from build123d import *

# Parameters (mm, degrees)
SKETCH_1_W             = 90
SKETCH_1_H             = 75
SKETCH_1_R             = 26
EXTRUDE_1_DEPTH        = 30
HOLE_WIZARD_M8_1_D     = 6.8
HOLE_WIZARD_M8_1_DEPTH = 19.75
HOLE_WIZARD_M8_1_TIP   = 2.042926105
CHAMFER_1_SIZE         = 15
HOLE_WIZARD_M8_2_D     = 6.8
HOLE_WIZARD_M8_2_DEPTH = 19.75
HOLE_WIZARD_M8_2_TIP   = 2.042926105


with BuildPart() as part:
    # 草图1 → 凸台-拉伸1 (new, symmetric)
    with BuildSketch(Plane.XY):
        with Locations((0, 5)):
            Rectangle(SKETCH_1_W, SKETCH_1_H)
        Circle(SKETCH_1_R, mode=Mode.SUBTRACT)
    extrude(amount=EXTRUDE_1_DEPTH, both=True)

    # M8 螺纹孔1
    with Locations(Plane(origin=(-32.5, 0, 30), x_dir=(1, 0, 0), z_dir=(0, 0, 1))):
        with Locations((0, 0), (9.519029611, 22.980970389), (9.519029611, -22.980970389), (55.480970389, -22.980970389), (65, 0), (55.480970389, 22.980970389)):
            Hole(HOLE_WIZARD_M8_1_D / 2, depth=HOLE_WIZARD_M8_1_DEPTH)
            with Locations((0, 0, -(HOLE_WIZARD_M8_1_DEPTH + HOLE_WIZARD_M8_1_TIP / 2))):  # 118° drill point
                Cone(0, HOLE_WIZARD_M8_1_D / 2, HOLE_WIZARD_M8_1_TIP, mode=Mode.SUBTRACT)

    # 倒角1
    chamfer_1_edges = [part.edges().sort_by_distance(p)[0] for p in [
        (45, -32.5, 0),
        (-45, -32.5, 0),
    ]]
    chamfer(chamfer_1_edges, length=CHAMFER_1_SIZE)

    # M8 螺纹孔2
    with Locations(Plane(origin=(32.5, 42.5, -20), x_dir=(1, 0, 0), z_dir=(0, 1, 0))):
        with Locations((0, 0), (0, -40), (-65, -40), (-65, 0)):
            Hole(HOLE_WIZARD_M8_2_D / 2, depth=HOLE_WIZARD_M8_2_DEPTH)
            with Locations((0, 0, -(HOLE_WIZARD_M8_2_DEPTH + HOLE_WIZARD_M8_2_TIP / 2))):  # 118° drill point
                Cone(0, HOLE_WIZARD_M8_2_D / 2, HOLE_WIZARD_M8_2_TIP, mode=Mode.SUBTRACT)


solid = part.part
Input: part model. Units: mm. Frame: model coordinates. A direction names the side the tool comes from. Coordinates: 2 decimals unless noted, no trailing zeros. Write each loop counter-clockwise with the first axis right and the second up, starting at its lowest first coordinate (ties: lowest second). Pieces come first, ordered by that corner, then holes. Notation, with made-up numbers: M 39,70.25 L 73,70.25 A7 ccw 73,75.25 Z; hole C -22.5,15 d11. An arc over 180 degrees is marked long. Answer as a JSON object with one key per item and string values. Group by question number.
(1) Section A-A on x = 0. Output: boundary loops of the cut face in (y, z), plus the area to 3 significant figures.
(2) Section B-B on y = 33.5. Output: boundary loops of the cut face in (x, z).
(3) Mould query, pull axis X, two halves, no side actions, for faces 1 (the face through (-37.4, -25.1, -0.4)), 2 (the face through (-31.94, 0.18, 8.56)), 3 (the face through (37.6, -24.9, -0.4)). Classes: pulls with the +X half, pulls with the -X half, needs draft (parallel to the pull), parting line crosses it, or undercut.
(4) Set-up query: faces 4 (the face through (-20.633, -15.821, -0.42)), 5 (the face through (-35.64, -1.3, 19.99)), 6 (the face through (29.36, 32.49, -18.7)). Return all of +Z, -Z, +X, -X, +Y, -Y with unobstructed straight access to the full face (end or side cutting, diameter ignored); none if empty.
(5) Contact query for flat-ended pins moving along their axis: P1, Ø5.5, axis at x = -22.98, y = 22.98, coming from the +Z side; P2, Ø5.5, axis at x = 32.5, z = 20, coming from the +Y side; P3, Ø6, axis at x = -32.5, z = -20, coming from the +Y side. Output: stop coordinate, or through.
(6) Section D-D on y = -11.5. Output: boundary loops of the cut face in (x, z), plus the area to 3 significant figures.
(7) Section C-C on z = 3. Output: boundary loops of the cut face in (x, y).
(8) Ray query, line 1 along X through (y, z) = (32, -20); line 2 along Y through (x, z) = (0.5, 20); line 3 along Z through (x, y) = (32, 30). Return the intervals inside material, ascending. Write a range as [from, to].
Result set:
{
 "1": {"outline": "M -32.5,-30 L -26,-30 L -26,30 L -32.5,30 Z; M 26,-30 L 42.5,-30 L 42.5,30 L 26,30 Z", "area": "1,380 mm2"},
 "2": {"outline": "M -45,-30 L 45,-30 L 45,30 L -45,30 Z; hole C -32.5,-20 d6.8; hole C -32.5,20 d6.8; hole C 32.5,-20 d6.8; hole C 32.5,20 d6.8"},
 "3": {"face 1": "pulls with the -X half", "face 2": "undercut", "face 3": "pulls with the +X half"},
 "4": {"face 4": "+Z, -Z", "face 5": "+Z", "face 6": "+Y"},
 "5": {"P1": "stops at z = 9.86", "P2": "stops at y = 22.36", "P3": "stops at y = 22.51"},
 "6": {"outline": "M -45,-30 L -23.32,-30 L -23.32,30 L -45,30 Z; M 23.32,-30 L 45,-30 L 45,30 L 23.32,30 Z", "area": "2,600 mm2"},
 "7": {"outline": "M -45,-17.5 L -30,-32.5 L 30,-32.5 L 45,-17.5 L 45,42.5 L -45,42.5 Z; hole C 0,0 d52"},
 "8": {"line 1": "x = [-45, -35.9], [-29.1, 29.1], [35.9, 45]", "line 2": "y = [-32.5, -26], [26, 42.5]", "line 3": "z = [-30, -23.36], [-16.64, 16.64], [23.36, 30]"}
}
